Verification items for the finished model (mm, model axes). Round coordinates to 2 decimals unless told otherwise and drop trailing zeros. Loops run counter-clockwise (first coordinate to the right, second up) from the corner with the lowest first, then second, coordinate; pieces in that order, holes last. Notation, with made-up numbers: M 39.25,-5 L 54.25,-5 A19 cw 54.25,2 Z; hole C 59,32 d1. An arc over 180 degrees is marked long. Answer as CSV lines item,"result".
```python
from build123d import *

# Parameters (mm, degrees)
BASENUT_START = -44.6786
BASENUTSKE_R  = 19.84375
BASENUT_DEPTH = 44.6786


with BuildPart() as part:
    # BaseNutSke → BaseNut (new body)
    with BuildSketch(Plane.XY.offset(BASENUT_START)):
        Polygon((34.925, 20.163958151), (34.925, -20.163958151), (0, -40.327916303), (-34.925, -20.163958151), (-34.925, 20.163958151), (0, 40.327916303), align=None)
        Circle(BASENUTSKE_R, mode=Mode.SUBTRACT)
    extrude(amount=BASENUT_DEPTH)

    # Sketch3 → Double-Chamfer (revolve, cut)
    with BuildSketch(Plane(origin=(0, 0, 0), x_dir=(0, 0, -1), z_dir=(1, 0, 0))):
        Polygon((44.6786, 34.925), (40.2336, 40.327916303), (40.2336, 53.027916303), (57.3786, 53.027916303), (57.3786, 34.925), align=None)
        Polygon((4.445, 53.027916303), (-12.7, 53.027916303), (-12.7, 34.925), (0, 34.925), (4.445, 40.327916303), align=None)
    revolve(axis=Axis((0, 0, 0), (0, 0, -1)), mode=Mode.SUBTRACT)

    # Sketch5 → EndChamfer (revolve, cut)
    with BuildSketch(Plane(origin=(0, 0, 0), x_dir=(0, 0, -1), z_dir=(1, 0, 0)), mode=Mode.PRIVATE) as endchamfer_sk:
        Polygon((44.6532, 22.225), (42.81909388, 19.605625), (44.704, 19.605625), (44.704, 22.225), align=None)
        Polygon((-0.0508, 22.225), (0, 22.225), (1.83410612, 19.605625), (-0.0508, 19.605625), align=None)
    revolve(endchamfer_sk.sketch.rotate(Axis((0, 0, -25.037505729), (0, 0, -1)), 90), axis=Axis((0, 0, -25.037505729), (0, 0, -1)), mode=Mode.SUBTRACT)


solid = part.part
```
1) Material ranges on probe 1 along X at (y, z) = (12, -24) (3 decimals); probe 2 along X at (y, z) = (14, -34) (3 decimals); probe 3 along Y at (x, z) = (-4, -29), recorded low to high.
Here are the results:
probe 1,"x = -34.925 to -15.804, 15.804 to 34.925"
probe 2,"x = -34.925 to -14.063, 14.063 to 34.925"
probe 3,"y = -38.02 to -19.44, 19.44 to 38.02"
2) Go/stop test with flat-tipped pins: pin 1 (6 mm diameter, centred on y = -21, z = -12.5, fed in from -X) (3 decimals); pin 2 (2 mm diameter, centred on x = 26.5, z = -22, fed in from +Y); pin 3 (3 mm diameter, centred on x = -2.5, z = -27, fed in from -Y); pin 4 (10 mm diameter, centred on x = -18.5, z = -23.5, fed in from -Y). Record where each tip stops, or that it passes through.
Here are the results:
pin 1,"stops at x = -34.925"
pin 2,"stops at y = 25.61"
pin 3,"stops at y = -39.75"
pin 4,"stops at y = -32.53"
3) Section check A-A (z = -21.5). Record the cut outline in (x, y) (1 decimal).
Here are the results:
outline,"M -34.9,-20.2 L 0,-40.3 L 34.9,-20.2 L 34.9,20.2 L 0,40.3 L -34.9,20.2 Z; hole C 0,0 d39.7"
4) Draft check along Y on faces 1 (the conical face through (31.427, -18.042, -43.598)), 2 (the cylindrical face through (18.927, 5.961, -22.616)), 3 (the flat face through (-17.707, 30.105, -22.652)), 4 (the flat face through (34.925, 0, -23)). Enter one of: +Y half, -Y half, draft (parallel to the pull), parting line (faces both ways), or undercut.
Here are the results:
face 1,"-Y half"
face 2,"undercut"
face 3,"+Y half"
face 4,"draft"
